The drawing under review shows one solid part. Ordinate dimensions are in mm from its lowest x, y, z. A direction names the side the tool comes from. Coordinates: 2 decimals unless noted, no trailing zeros. Write each loop counter-clockwise with the first axis right and the second up, starting at its lowest first coordinate (ties: lowest second). Pieces come first, ordered by that corner, then holes. Notation, with made-up numbers: (-24.75, 8) - (13.25, 8) arc R15 ccw to (13.25, 25) - close; hole circle Ø6 at (-10, -8.5). An arc over 180 degrees is marked (long way). Put each result on its own line as item: value. Start each with the question number.
Item 1: Consider section B-B on x = 35. Give the boundary of the cut face in (y, z), then the cut area to 3 significant figures.
Item 2: Consider section D-D on y = 48.5. Give the boundary of the cut face in (x, z).
Item 3: Consider section C-C on x = 72.5. Give the boundary of the cut face in (y, z), then the cut area to 4 significant figures.
Item 4: Machinability: for the marked faces 1 and 2, which of the approach directions +Z, -Z, +X, -X, +Y, -Y give a long, thin tool a straight path to every point of the face, cutting with its end or side? Answer none if there is none.
Item 5: To check wall thickness, follow L1, parallel to Y at x = 35, z = 11; L2, parallel to Y at x = 12, z = 16.85; L3, parallel to X at y = 6, z = 17.5. State the ranges of each line that lie inside material, in increasing order. Write a range as [from, to].
Item 6: Consider section A-A on y = 12. Give the boundary of the cut face in (x, z).
Item 7: For pin 1 (9 mm diameter, centred on x = 35, y = 12, fed in from +Z); pin 2 (4 mm diameter, centred on y = 17, z = 5.5, fed in from -X), all flat-tipped, find the tip position at first contact; note any pin that passes through.
Item 8: Mouldability with a two-part tool opening along X and no side actions: class the marked faces 3, 4 and 5 as pulls with the +X half, pulls with the -X half, needs draft (parallel to the pull), parting line crosses it, or undercut.
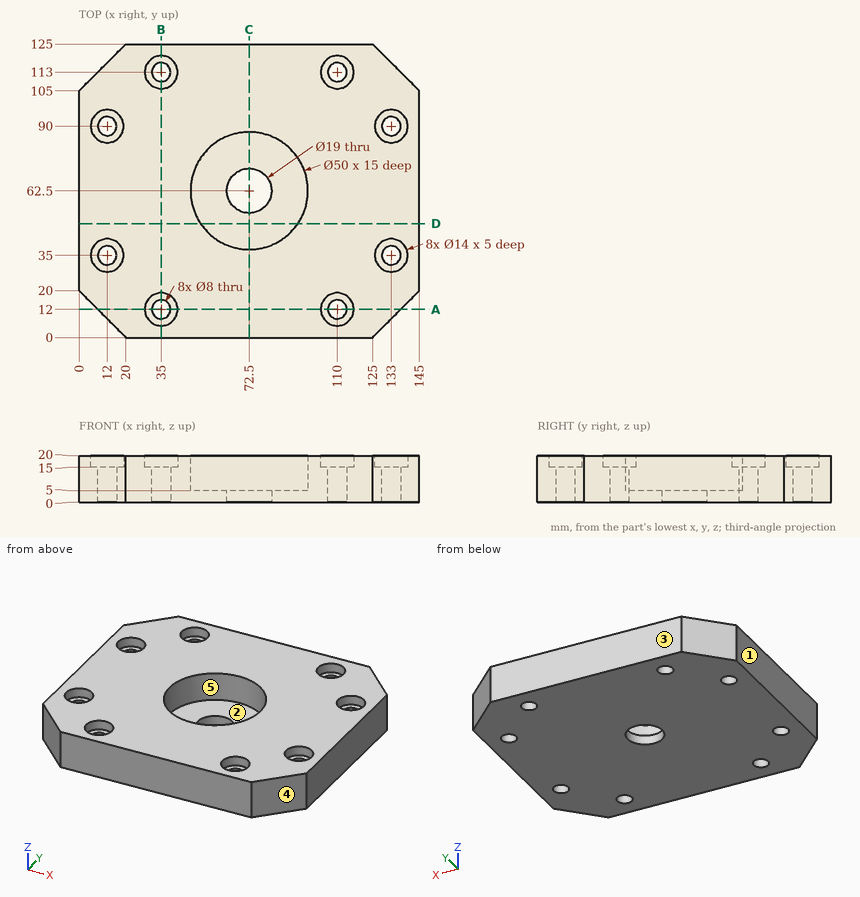
Report:
1. outline: (0, 0) - (8, 0) - (8, 15) - (5, 15) - (5, 20) - (0, 20) - close; (16, 0) - (109, 0) - (109, 15) - (106, 15) - (106, 20) - (19, 20) - (19, 15) - (16, 15) - close; (117, 0) - (125, 0) - (125, 20) - (120, 20) - (120, 15) - (117, 15) - close
1. area: 2,120 mm²
2. outline: (0, 0) - (145, 0) - (145, 20) - (93.21, 20) - (93.21, 5) - (51.79, 5) - (51.79, 20) - (0, 20) - close
3. outline: (0, 0) - (53, 0) - (53, 5) - (37.5, 5) - (37.5, 20) - (0, 20) - close; (72, 0) - (125, 0) - (125, 20) - (87.5, 20) - (87.5, 5) - (72, 5) - close
3. area: 1,655 mm²
4. face 1: +Z, -Z, -X, +Y, -Y
4. face 2: +Z
5. L1: [0, 8], [16, 109], [117, 125]
5. L2: [8, 28], [42, 83], [97, 117]
5. L3: [14, 31.39], [38.61, 106.39], [113.61, 131]
6. outline: (8, 0) - (31, 0) - (31, 15) - (28, 15) - (28, 20) - (8, 20) - close; (39, 0) - (106, 0) - (106, 15) - (103, 15) - (103, 20) - (42, 20) - (42, 15) - (39, 15) - close; (114, 0) - (137, 0) - (137, 20) - (117, 20) - (117, 15) - (114, 15) - close
7. pin 1: z = 15
7. pin 2: x = 1
8. face 3: needs draft
8. face 4: pulls with the +X half
8. face 5: undercut
